from build123d import *

# Parameters (mm, degrees)
BOSS_EXTRUDE1_DEPTH      = 5
BOSS_EXTRUDE1_DEPTH_BACK = 5
BOSS_EXTRUDE2_DEPTH      = 1
SKETCH3_W                = 100
SKETCH3_H                = 100
SKETCH3_R                = 20.87
CUT_EXTRUDE1_DEPTH       = 2


with BuildPart() as part:
    # Sketch1 → Boss-Extrude1 (new, two sides: drawn at the far end of the back side and taken through both)
    with BuildSketch(Plane.XY.offset(-BOSS_EXTRUDE1_DEPTH_BACK)):
        with BuildLine():
            Line((0, 0), (10.5, 0))
            ThreePointArc((10.5, 0), (12.813469706, 1.552446351), (12.253709329, 4.281713666))
            Line((12.253709329, 4.281713666), (10, 6.5))
            Line((10, 6.5), (9.298516268, 5.787314534))
            Line((9.298516268, 5.787314534), (11.552225598, 3.5690282))
            ThreePointArc((11.552225598, 3.5690282), (11.888081824, 1.931467811), (10.5, 1))
            Line((10.5, 1), (0, 1))
            Line((0, 1), (0, 0))
        make_face()
    extrude(amount=BOSS_EXTRUDE1_DEPTH + BOSS_EXTRUDE1_DEPTH_BACK)

    # Sketch2 → Boss-Extrude2 (add)
    with BuildSketch(Plane(origin=(0, 0, 0), x_dir=(1, 0, 0), z_dir=(0, 1, 0))):
        with BuildLine():
            Line((3.134247972, -11), (11.75, -11))
            ThreePointArc((11.75, -11), (13.5, -9.25), (11.75, -7.5))
            Line((11.75, -7.5), (11.69, -7.5))
            ThreePointArc((11.69, -7.5), (11.124314575, -7.265685425), (10.89, -6.7))
            Line((10.89, -6.7), (10.89, 6.7))
            ThreePointArc((10.89, 6.7), (11.124314575, 7.265685425), (11.69, 7.5))
            Line((11.69, 7.5), (11.75, 7.5))
            ThreePointArc((11.75, 7.5), (13.5, 9.25), (11.75, 11))
            Line((11.75, 11), (3.134247972, 11))
            ThreePointArc((3.134247972, 11), (0, 0), (3.134247972, -11))
        make_face()
    extrude(amount=BOSS_EXTRUDE2_DEPTH)

    # Sketch3 → Cut-Extrude1 (cut)
    with BuildSketch(Plane(origin=(0, 0, 0), x_dir=(1, 0, 0), z_dir=(0, 1, 0))):
        Rectangle(SKETCH3_W, SKETCH3_H)
        with Locations((20.87, 0)):
            Circle(SKETCH3_R, mode=Mode.SUBTRACT)
    extrude(amount=CUT_EXTRUDE1_DEPTH, mode=Mode.SUBTRACT)

    # Sketch4 → Cut-Revolve1 (revolve, cut)
    with BuildSketch(Plane.XY.offset(6.75), mode=Mode.PRIVATE) as cut_revolve1_sk:
        Polygon((7, 1), (9.1, 1), (8.6, 0), (7, 0), align=None)
    revolve(cut_revolve1_sk.sketch.rotate(Axis((7, 0, 6.75), (0, 1, 0)), 270), axis=Axis((7, 0, 6.75), (0, 1, 0)), mode=Mode.SUBTRACT)

    # Sketch5 → Cut-Revolve2 (revolve, cut)
    with BuildSketch(Plane.XY.offset(-6.75), mode=Mode.PRIVATE) as cut_revolve2_sk:
        Polygon((7, 1), (9.1, 1), (8.6, 0), (7, 0), align=None)
    revolve(cut_revolve2_sk.sketch.rotate(Axis((7, 0, -6.75), (0, 1, 0)), 270), axis=Axis((7, 0, -6.75), (0, 1, 0)), mode=Mode.SUBTRACT)


solid = part.part
Part model, mm, in its own coordinate system. A direction names the side the tool comes from. Coordinates: 2 decimals unless noted, no trailing zeros. Order: outer loops, then holes, each group sorted by start corner. A loop starts at its lowest first (then second) coordinate and runs counter-clockwise, first axis right, second up.
(1) Slice it at C-C, the plane y = 2.5. Write the cut outline in (x, z), and give its area (4 significant figures).
Check sheet entries:
outline: (12, -5) - (13, -5) - (13, 5) - (12, 5) - close
area: 10.00 mm2
(2) Tool access for faces 1 (the face through (12.87, 1.7, -0.07)), 2 (the face through (12, 4, 5)), 3 (the face through (10.41, 4.694, -0.07)): list every direction of +Z, -Z, +X, -X, +Y, -Y with a clear straight run to the whole face (end or side of a thin tool).
Check sheet entries:
face 1: +X
face 2: +X, +Y
face 3: +Z, -Z, -X
(3) Probe L1, parallel to Y at x = 5.25, z = 9.5; L2, parallel to X at y = 4, z = 4; L3, parallel to Z at x = 2.25, y = 0.5. List the from-to ranges inside material, lowest first.
Check sheet entries:
L1: y = 0 to 1
L2: x = 11.11 to 12.5
L3: z = -9.43 to 9.43
(4) Pin check, flat tips, straight feed: pin 1 Ø1.5 at (x, z) = (11, -6.5) entering from +Y; pin 2 Ø1 at (y, z) = (2.5, -3) entering from +X; pin 3 Ø1.9 at (x, y) = (11, 2) entering from -Z; pin 4 Ø1 at (x, y) = (2.5, 2.5) entering from -Z. Stop position of each tip, or through.
Check sheet entries:
pin 1: stops at y = 1
pin 2: stops at x = 13
pin 3: stops at z = -5
pin 4: passes through
(5) Slice it at A-A, the plane x = 7. Write the cut outline in (y, z).
Check sheet entries:
outline: (0, -11) - (1, -11) - (1, -8.85) - (0, -8.35) - close; (0, -5.15) - (1, -4.65) - (1, 4.65) - (0, 5.15) - close; (0, 8.35) - (1, 8.85) - (1, 11) - (0, 11) - close
